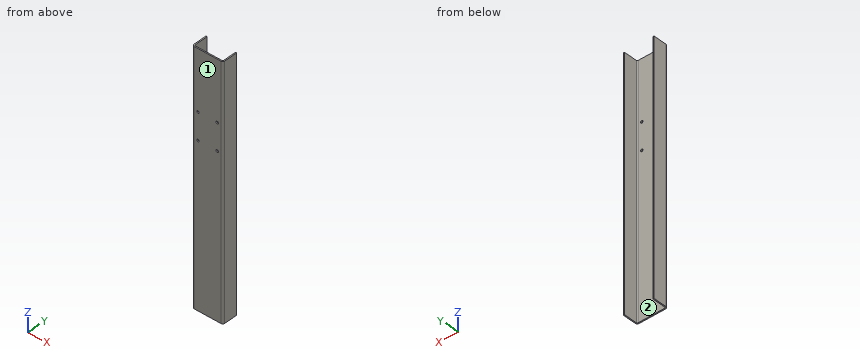
from build123d import *

# Parameters (mm, degrees)
BOSS_EXTRUDE1_DEPTH = 645
SKETCH2_R           = 3.25
CUT_EXTRUDE1_DEPTH  = 10


with BuildPart() as part:
    # Sketch1 → Boss-Extrude1 (new body)
    with BuildSketch(Plane.XY):
        with BuildLine():
            Line((0, 0), (0, -35))
            ThreePointArc((0, -35), (1.464466094, -38.535533906), (5, -40))
            Line((5, -40), (75, -40))
            ThreePointArc((75, -40), (78.535533906, -38.535533906), (80, -35))
            Line((80, -35), (80, 0))
            Line((80, 0), (77, 0))
            Line((77, 0), (77, -35))
            ThreePointArc((77, -35), (76.414213562, -36.414213562), (75, -37))
            Line((75, -37), (5, -37))
            ThreePointArc((5, -37), (3.585786438, -36.414213562), (3, -35))
            Line((3, -35), (3, 0))
            Line((3, 0), (0, 0))
        make_face()
    extrude(amount=BOSS_EXTRUDE1_DEPTH)

    # Sketch2 → Cut-Extrude1 (cut)
    with BuildSketch(Plane.XZ.offset(40)):
        with Locations(Location((15, 489, 0), (0, 0, 270))):
            Circle(SKETCH2_R)
        with Locations(Location((65, 489, 0), (0, 0, 270))):
            Circle(SKETCH2_R)
        with Locations(Location((15, 419, 0), (0, 0, 270))):
            Circle(SKETCH2_R)
        with Locations(Location((65, 419, 0), (0, 0, 270))):
            Circle(SKETCH2_R)
    extrude(amount=-CUT_EXTRUDE1_DEPTH, mode=Mode.SUBTRACT)


solid = part.part
Geometry check sheet. Reference: the model listing, model coordinates, mm. Face numbers are marked on the shaded views. Give positions to 0.01 mm unless a question says otherwise; leave off trailing zeros. Order: outer loops, then holes, each group sorted by start corner. A loop starts at its lowest first (then second) coordinate and runs counter-clockwise, first axis right, second up.
1) Cross-section at B-B (z = 477.5). Record the boundary of the cut face in (x, y), then the cut area to 3 significant figures.
Results are:
outline: (0, -35) arc R5 ccw to (5, -40) - (75, -40) arc R5 ccw to (80, -35) - (80, 0) - (77, 0) - (77, -35) arc R2 cw to (75, -37) - (5, -37) arc R2 cw to (3, -35) - (3, 0) - (0, 0) - close
area: 453 mm2
2) Cross-section at A-A (y = -25.5). Record the boundary of the cut face in (x, z), then the cut area to 3 significant figures.
Results are:
outline: (0, 0) - (3, 0) - (3, 645) - (0, 645) - close; (77, 0) - (80, 0) - (80, 645) - (77, 645) - close
area: 3,870 mm2
3) Gauge pin test, flat end, axial feed: pin 1 (7.5 mm diameter, centred on x = 65, z = 419, fed in from +Y). Record the tip position at first contact, or that the pin passes through.
Results are:
pin 1: stops at y = -37
4) Material ranges on probe 1 along X at (y, z) = (-29.5, 325); probe 2 along X at (y, z) = (-39, 419); probe 3 along Y at (x, z) = (55.5, 115), recorded low to high.
Results are:
probe 1: x = 0 to 3, 77 to 80
probe 2: x = 2 to 11.75, 18.25 to 61.75, 68.25 to 78
probe 3: y = -40 to -37
5) Draft check along X on the marked faces 1 and 2. Enter one of: released by +X, released by -X, zero draft, split by the parting line, or undercut.
Results are:
face 1: zero draft
face 2: undercut
6) Cross-section at C-C (x = 44). Record the boundary of the cut face in (y, z).
Results are:
outline: (-40, 0) - (-37, 0) - (-37, 645) - (-40, 645) - close
